from build123d import *

# Parameters (mm, degrees)
SKETCH_1_W               = 34
SKETCH_1_H               = 19.5
EXTRUDE_1_DEPTH          = 28.4
CUT_EXTRUDE_1_DEPTH      = 35.505398128
CUT_EXTRUDE_1_DEPTH_BACK = 35.505398128
SKETCH_2_W               = 15
SKETCH_2_H               = 8
SKETCH_4_R               = 1.8
CUT_EXTRUDE_2_DEPTH      = 6


with BuildPart() as part:
    # 草图1 → 凸台-拉伸1 (new, symmetric)
    with BuildSketch(Plane.XY):
        Rectangle(SKETCH_1_W, SKETCH_1_H)
    extrude(amount=EXTRUDE_1_DEPTH, both=True)

    # 草图2 → 切除-拉伸1 (cut, two sides: drawn at the far end of the back side and taken through both)
    with BuildSketch(Plane.XY.offset(-CUT_EXTRUDE_1_DEPTH_BACK)):
        with Locations((0, -5.75)):
            Rectangle(SKETCH_2_W, SKETCH_2_H)
    extrude(amount=CUT_EXTRUDE_1_DEPTH + CUT_EXTRUDE_1_DEPTH_BACK, mode=Mode.SUBTRACT)

    # 草图4 → 切除-拉伸2 (cut)
    with BuildSketch(Plane(origin=(0, 9.75, 0), x_dir=(1, 0, 0), z_dir=(0, 1, 0))):
        with Locations(Location((-13, 13, 0), (0, 0, 270))):
            Circle(SKETCH_4_R)
        with Locations(Location((13, 13, 0), (0, 0, 90))):
            Circle(SKETCH_4_R)
        with Locations(Location((13, -13, 0), (0, 0, 270))):
            Circle(SKETCH_4_R)
        with Locations(Location((-13, -13, 0), (0, 0, 90))):
            Circle(SKETCH_4_R)
    extrude(amount=-CUT_EXTRUDE_2_DEPTH, mode=Mode.SUBTRACT)


solid = part.part
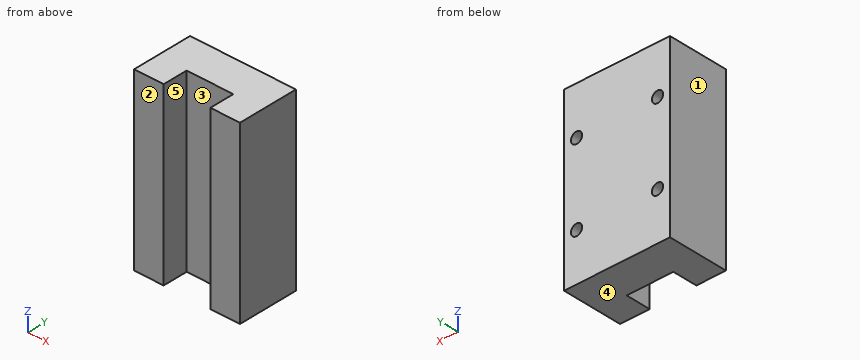
Read the model definition and answer for the solid it produces. Units are mm, in the model's axes. Face numbers are marked on the shaded views. A direction names the side the tool comes from. Coordinates: 2 decimals unless noted, no trailing zeros. Loops run counter-clockwise (first coordinate to the right, second up) from the corner with the lowest first, then second, coordinate; pieces in that order, holes last. Notation, with made-up numbers: (-11.75, -29.5) - (6.25, -29.5) arc R27 cw to (6.25, -5.5) - close; hole circle Ø3 at (50, 61.5). An arc over 180 degrees is marked (long way). Answer in a Markdown table with one row per item.
Q1. Find section A-A on y = -6.25. Write down the section's boundary in (x, z), plus the area to 3 significant figures.
Here are the results:
| item | result |
|---|---|
| outline | (-17, -28.4) - (-7.5, -28.4) - (-7.5, 28.4) - (-17, 28.4) - close; (7.5, -28.4) - (17, -28.4) - (17, 28.4) - (7.5, 28.4) - close |
| area | 1,080 mm^2 |
Q2. Given P1, Ø7.5, axis at x = 3, z = 10, coming from the -Y side; P2, Ø1.1, axis at x = 13.5, z = 14, coming from the +Y side, each flat-ended and moving along its own axis, determine where each tip first touches the part or whether it passes through.
Here are the results:
| item | result |
|---|---|
| P1 | stops at y = -1.75 |
| P2 | stops at y = 3.75 |
Q3. The mould has two halves that part along X. Classify the marked faces 1, 2 and 3: pulls with the +X half, pulls with the -X half, needs draft (parallel to the pull), parting line crosses it, or undercut.
Here are the results:
| item | result |
|---|---|
| face 1 | pulls with the -X half |
| face 2 | needs draft |
| face 3 | undercut |
Q4. Straight lines are drawn through the part: line 1 along X through (y, z) = (5.9, 13); line 2 along X through (y, z) = (-3.5, -16.5); line 3 along Y through (x, z) = (6, 14.5). For each, find the intervals that lie inside material, in ascending order. Write a range as [from, to].
Here are the results:
| item | result |
|---|---|
| line 1 | x = [-17, -14.8], [-11.2, 11.2], [14.8, 17] |
| line 2 | x = [-17, -7.5], [7.5, 17] |
| line 3 | y = [-1.75, 9.75] |
Q5. Find section C-C on x = 13. Write down the section's boundary in (y, z).
Here are the results:
| item | result |
|---|---|
| outline | (-9.75, -28.4) - (9.75, -28.4) - (9.75, -14.8) - (3.75, -14.8) - (3.75, -11.2) - (9.75, -11.2) - (9.75, 11.2) - (3.75, 11.2) - (3.75, 14.8) - (9.75, 14.8) - (9.75, 28.4) - (-9.75, 28.4) - close |
Q6. Find section B-B on y = 6.5. Write down the section's boundary in (x, z).
Here are the results:
| item | result |
|---|---|
| outline | (-17, -28.4) - (17, -28.4) - (17, 28.4) - (-17, 28.4) - close; hole circle Ø3.6 at (-13, -13); hole circle Ø3.6 at (-13, 13); hole circle Ø3.6 at (13, -13); hole circle Ø3.6 at (13, 13) |
Q7. Find section D-D on z = 13. Write down the section's boundary in (x, y), plus the area to 3 significant figures.
Here are the results:
| item | result |
|---|---|
| outline | (-17, -9.75) - (-7.5, -9.75) - (-7.5, -1.75) - (7.5, -1.75) - (7.5, -9.75) - (17, -9.75) - (17, 9.75) - (14.8, 9.75) - (14.8, 3.75) - (11.2, 3.75) - (11.2, 9.75) - (-11.2, 9.75) - (-11.2, 3.75) - (-14.8, 3.75) - (-14.8, 9.75) - (-17, 9.75) - close |
| area | 500 mm^2 |
Q8. For the marked faces 4 and 5, determine the directions among +Z, -Z, +X, -X, +Y, -Y from which every point of the face is accessible in a straight line to the end or side of a thin tool.
Here are the results:
| item | result |
|---|---|
| face 4 | -Z, +X, -X, +Y, -Y |
| face 5 | +Z, -Z, -Y |
